Geometry check sheet. Reference: the model listing, model coordinates, mm. A direction names the side the tool comes from. Coordinates: 2 decimals unless noted, no trailing zeros. Write each loop counter-clockwise with the first axis right and the second up, starting at its lowest first coordinate (ties: lowest second). Pieces come first, ordered by that corner, then holes. Notation, with made-up numbers: M 24.5,29 L 81.5,29 A15 ccw 81.5,34 Z; hole C -11,46 d1. An arc over 180 degrees is marked long. Put each result on its own line as item: value. Start each with the question number.
1) Scan lines: line 1 along X through (y, z) = (121, 31.5); line 2 along Z through (x, y) = (0, 176); line 3 along X through (y, z) = (188, 80). Record each from-to range of solid material in increasing order.
2) Gauge pin test, flat ends, axial feed: pin 1 (15.5 mm diameter, centred on x = -256, z = 18.5, fed in from -Y); pin 2 (15.5 mm diameter, centred on x = 130.5, z = 8, fed in from +Y); pin 3 (5 mm diameter, centred on x = -7.5, y = 167.5, fed in from +Z). Record the tip position at first contact, or that the pin passes through.
3) Cross-section at D-D on y = 27.5. Record the cut outline in (x, z), plus the area to 3 significant figures.
4) Cross-section at C-C on z = 36. Count the separate pieces of the cut face and the enclosed holes in it, plus the area to 3 significant figures.
5) Mould release check, pull along X, two halves, no side actions. Record for faces 6 (the flat face through (-283.95, 115.7, 35.775)), 7 (the flat face through (5.6, 27.14, 127.92)), 8 (the flat face through (-400, 33, 65)): released by +X, released by -X, zero draft, split by the parting line, or undercut.
6) Cross-section at B-B on y = 89. Record the cut outline in (x, z), plus the area to 3 significant figures.
7) Set-up check for faces 1 (the conical face through (377.04, 130.18, 46.43)), 2 (the flat face through (5.53, 106.307, 85.296)), 3 (the flat face through (-94, 165, 26)), 4 (the cylindrical face through (0.38, 186.56, 88.74)), 5 (the flat face through (325, 200, 165)): record each of +Z, -Z, +X, -X, +Y, -Y from which the full face is reachable in a straight line by a thin tool's end or side.
8) Cross-section at A-A on x = -65. Record the cut outline in (y, z), plus the area to 3 significant figures.
from build123d import *

# Parameters (mm, degrees)
BOSS_EXTRUDE1_DEPTH                    = 400
SKETCH3_W                              = 720
SKETCH3_H                              = 10
CUT_EXTRUDE1_DEPTH                     = 487.672374396
CUT_EXTRUDE2_DEPTH                     = 325
CUT_EXTRUDE3_DEPTH                     = 650
SKETCH7_W                              = 10
SKETCH7_H                              = 100
CUT_EXTRUDE4_DEPTH                     = 650
BOSS_EXTRUDE2_REACH                    = 488.672
SKETCH8_W                              = 40
SKETCH8_H                              = 100
SKETCH8_W_2                            = 35
M20_TAPPED_HOLE1_D                     = 17.5
M20_TAPPED_HOLE1_DEPTH                 = 45
M20_TAPPED_HOLE1_CSINK_D               = 20.05
M20_TAPPED_HOLE1_CSINK_ANGLE           = 90
M20_TAPPED_HOLE1_TIP                   = 5.257530416
M20_TAPPED_HOLE2_D                     = 17.5
M20_TAPPED_HOLE2_DEPTH                 = 40
M20_TAPPED_HOLE2_CSINK_D               = 20.05
M20_TAPPED_HOLE2_CSINK_ANGLE           = 90
M20_TAPPED_HOLE2_TIP                   = 5.257530416
M20_TAPPED_HOLE2_ON_FACE_2_D           = 17.5
M20_TAPPED_HOLE2_ON_FACE_2_DEPTH       = 40
M20_TAPPED_HOLE2_ON_FACE_2_CSINK_D     = 20.05
M20_TAPPED_HOLE2_ON_FACE_2_CSINK_ANGLE = 90
M20_TAPPED_HOLE2_ON_FACE_2_TIP         = 5.257530416
FILLET1_R                              = 10


with BuildPart() as part:
    # Sketch1 → Boss-Extrude1 (new, symmetric)
    with BuildSketch(Plane(origin=(0, 0, 0), x_dir=(0, 0, -1), z_dir=(1, 0, 0))):
        Polygon((0, 0), (-119.1, 0), (-131.429467258, 37.946198403), (-73.515136927, 70.048635914), (-102.788489796, 160.142752116), (-168.511506583, 152.072980358), (-175, 172.042509728), (-175, 215), (0, 215), (0, 165), (-51.793594091, 165), (-19.301624468, 65), (0, 65), align=None)
    extrude(amount=BOSS_EXTRUDE1_DEPTH, both=True)

    # Sketch3 → Cut-Extrude1 (cut, through all)
    with BuildSketch(Plane.XY):
        with Locations((0, 215)):
            Rectangle(SKETCH3_W, SKETCH3_H)
    extrude(amount=CUT_EXTRUDE1_DEPTH, mode=Mode.SUBTRACT)

    # Sketch4 → Cut-Extrude2 (cut, symmetric)
    with BuildSketch(Plane(origin=(0, 0, 0), x_dir=(0, 0, -1), z_dir=(1, 0, 0))):
        Polygon((-175, 215), (-175, 185), (-145, 215), align=None)
    extrude(amount=CUT_EXTRUDE2_DEPTH, both=True, mode=Mode.SUBTRACT)

    # Sketch6 → Cut-Extrude3 (cut)
    with BuildSketch(Plane(origin=(0, 0, 0), x_dir=(-1, 0, 0), z_dir=(0, 0, -1))):
        Polygon((-400, 0), (-360, 14.558809371), (-360, 19.558809371), (360, 19.558809371), (360, 14.558809371), (400, 0), align=None)
    extrude(amount=-CUT_EXTRUDE3_DEPTH, mode=Mode.SUBTRACT)

    # Sketch7 → Cut-Extrude4 (cut)
    with BuildSketch(Plane.XY):
        with Locations((-400, 115)):
            Rectangle(SKETCH7_W, SKETCH7_H)
    cut_extrude4 = extrude(amount=CUT_EXTRUDE4_DEPTH, mode=Mode.SUBTRACT)

    # Mirror1: Cut-Extrude4 across plane
    add(cut_extrude4.mirror(Plane(origin=(0, 0, 0), x_dir=(0, 0, 1), z_dir=(1, 0, 0))), mode=Mode.SUBTRACT)

    # Boss-Extrude2: up to this plane
    boss_extrude2_end = Plane(origin=(400, 165, 51.793594091), z_dir=(0, -0.309016994374942, 0.9510565162951553))
    # Sketch8 → Boss-Extrude2 (add, up to the surface)
    with BuildSketch(Plane(origin=(0, 0, 0), x_dir=(-1, 0, 0), z_dir=(0, 0, -1)), mode=Mode.PRIVATE) as boss_extrude2_sk1:
        with Locations((0, 115)):
            Rectangle(SKETCH8_W, SKETCH8_H)
    boss_extrude2_tool1 = split(extrude(boss_extrude2_sk1.sketch, amount=-BOSS_EXTRUDE2_REACH, mode=Mode.PRIVATE), bisect_by=boss_extrude2_end, keep=Keep.BOTH, mode=Mode.PRIVATE)
    add(boss_extrude2_tool1.solids().sort_by_distance((0, 115, 0))[0])
    # Sketch8 → Boss-Extrude2 (add, up to the surface)
    with BuildSketch(Plane(origin=(0, 0, 0), x_dir=(-1, 0, 0), z_dir=(0, 0, -1)), mode=Mode.PRIVATE) as boss_extrude2_sk2:
        with Locations((-190, 115)):
            Rectangle(SKETCH8_W, SKETCH8_H)
    boss_extrude2_tool2 = split(extrude(boss_extrude2_sk2.sketch, amount=-BOSS_EXTRUDE2_REACH, mode=Mode.PRIVATE), bisect_by=boss_extrude2_end, keep=Keep.BOTH, mode=Mode.PRIVATE)
    add(boss_extrude2_tool2.solids().sort_by_distance((190, 115, 0))[0])
    # Sketch8 → Boss-Extrude2 (add, up to the surface)
    with BuildSketch(Plane(origin=(0, 0, 0), x_dir=(-1, 0, 0), z_dir=(0, 0, -1)), mode=Mode.PRIVATE) as boss_extrude2_sk3:
        with Locations((190, 115)):
            Rectangle(SKETCH8_W, SKETCH8_H)
    boss_extrude2_tool3 = split(extrude(boss_extrude2_sk3.sketch, amount=-BOSS_EXTRUDE2_REACH, mode=Mode.PRIVATE), bisect_by=boss_extrude2_end, keep=Keep.BOTH, mode=Mode.PRIVATE)
    add(boss_extrude2_tool3.solids().sort_by_distance((-190, 115, 0))[0])
    # Sketch8 → Boss-Extrude2 (add, up to the surface)
    with BuildSketch(Plane(origin=(0, 0, 0), x_dir=(-1, 0, 0), z_dir=(0, 0, -1)), mode=Mode.PRIVATE) as boss_extrude2_sk4:
        with Locations((-377.5, 115)):
            Rectangle(SKETCH8_W_2, SKETCH8_H)
    boss_extrude2_tool4 = split(extrude(boss_extrude2_sk4.sketch, amount=-BOSS_EXTRUDE2_REACH, mode=Mode.PRIVATE), bisect_by=boss_extrude2_end, keep=Keep.BOTH, mode=Mode.PRIVATE)
    add(boss_extrude2_tool4.solids().sort_by_distance((377.5, 115, 0))[0])
    # Sketch8 → Boss-Extrude2 (add, up to the surface)
    with BuildSketch(Plane(origin=(0, 0, 0), x_dir=(-1, 0, 0), z_dir=(0, 0, -1)), mode=Mode.PRIVATE) as boss_extrude2_sk5:
        with Locations((377.5, 115)):
            Rectangle(SKETCH8_W_2, SKETCH8_H)
    boss_extrude2_tool5 = split(extrude(boss_extrude2_sk5.sketch, amount=-BOSS_EXTRUDE2_REACH, mode=Mode.PRIVATE), bisect_by=boss_extrude2_end, keep=Keep.BOTH, mode=Mode.PRIVATE)
    add(boss_extrude2_tool5.solids().sort_by_distance((-377.5, 115, 0))[0])

    # M20 Tapped Hole1
    with Locations(Plane(origin=(0, 210, 80), x_dir=(0, 0, 1), z_dir=(0, 1, 0))):
        with Locations((0, 0)):
            CounterSinkHole(M20_TAPPED_HOLE1_D / 2, M20_TAPPED_HOLE1_CSINK_D / 2, depth=M20_TAPPED_HOLE1_DEPTH, counter_sink_angle=M20_TAPPED_HOLE1_CSINK_ANGLE)
            with Locations((0, 0, -(M20_TAPPED_HOLE1_DEPTH + M20_TAPPED_HOLE1_TIP / 2))):  # 118° drill point
                Cone(0, M20_TAPPED_HOLE1_D / 2, M20_TAPPED_HOLE1_TIP, mode=Mode.SUBTRACT)

    # M20 Tapped Hole2
    with Locations(Plane(origin=(-377.5, 115.095694015, 88.151813362), x_dir=(0, 0.951056516295, 0.309016994375), z_dir=(0, -0.309016994375, 0.951056516295))):
        with Locations((0, 0)):
            CounterSinkHole(M20_TAPPED_HOLE2_D / 2, M20_TAPPED_HOLE2_CSINK_D / 2, depth=M20_TAPPED_HOLE2_DEPTH, counter_sink_angle=M20_TAPPED_HOLE2_CSINK_ANGLE)
            with Locations((0, 0, -(M20_TAPPED_HOLE2_DEPTH + M20_TAPPED_HOLE2_TIP / 2))):  # 118° drill point
                Cone(0, M20_TAPPED_HOLE2_D / 2, M20_TAPPED_HOLE2_TIP, mode=Mode.SUBTRACT)

    # M20 Tapped Hole2 on face 2
    with Locations(Plane(origin=(0, 115.095694015, 88.151813362), x_dir=(0, 0.951056560832, 0.309016857306), z_dir=(0, -0.309016857306, 0.951056560832))):
        with Locations((0, 0), (0, -377.5)):
            CounterSinkHole(M20_TAPPED_HOLE2_ON_FACE_2_D / 2, M20_TAPPED_HOLE2_ON_FACE_2_CSINK_D / 2, depth=M20_TAPPED_HOLE2_ON_FACE_2_DEPTH, counter_sink_angle=M20_TAPPED_HOLE2_ON_FACE_2_CSINK_ANGLE)
            with Locations((0, 0, -(M20_TAPPED_HOLE2_ON_FACE_2_DEPTH + M20_TAPPED_HOLE2_ON_FACE_2_TIP / 2))):  # 118° drill point
                Cone(0, M20_TAPPED_HOLE2_ON_FACE_2_D / 2, M20_TAPPED_HOLE2_ON_FACE_2_TIP, mode=Mode.SUBTRACT)

    # Fillet1
    fillet1_edges = [part.edges().sort_by_distance(p)[0] for p in [
        (0, 70.048635914, 73.515136927),
        (0, 160.142752116, 102.788489796),
    ]]
    fillet(fillet1_edges, radius=FILLET1_R)


solid = part.part
Answer key:
1. line 1: x = -395 to -360, -210 to -170, -20 to 20, 170 to 210, 360 to 395
1. line 2: z = 0 to 71.25, 88.75 to 175
1. line 3: x = -400 to -8.75, 8.75 to 400
2. pin 1: stops at y = 19.56
2. pin 2: stops at y = 210
2. pin 3: stops at z = 174.34
3. outline: M -400,0 L 400,0 L 400,128.04 L -400,128.04 Z
3. area: 102,000 mm²
4. separate pieces: 1
4. enclosed holes: 4
4. area: 124,000 mm²
5. face 6: undercut
5. face 7: zero draft
5. face 8: released by -X
6. outline: M -395,0 L -360,0 L -360,27.1 L -210,27.1 L -210,0 L -170,0 L -170,27.1 L -20,27.1 L -20,0 L 20,0 L 20,27.1 L 170,27.1 L 170,0 L 210,0 L 210,27.1 L 360,27.1 L 360,0 L 395,0 L 395,79.67 L -395,79.67 Z
6. area: 46,700 mm²
7. face 1: none
7. face 2: +Z, +X, -X
7. face 3: -Z
7. face 4: +Y
7. face 5: +Z, +Y
8. outline: M 19.56,0 L 65,0 L 65,19.3 L 165,51.79 L 165,0 L 210,0 L 210,150 L 185,175 L 172.04,175 L 152.07,168.51 L 159.14,110.97 A10 cw 152.3,100.24 L 77.89,76.06 A10 cw 66.05,80.72 L 37.95,131.43 L 19.56,125.46 Z
8. area: 18,700 mm²
